```python
from build123d import *

# Parameters (mm, degrees)
SKETCH1_R           = 127.5
SKETCH1_R_2         = 110
BOSS_EXTRUDE1_DEPTH = 5
SKETCH4_R           = 1
CUT_EXTRUDE2_DEPTH  = 5
CIRPATTERN2_COUNT   = 4


with BuildPart() as part:
    # Sketch1 → Boss-Extrude1 (new body)
    with BuildSketch(Plane.XY):
        Circle(SKETCH1_R)
        Circle(SKETCH1_R_2, mode=Mode.SUBTRACT)
    extrude(amount=BOSS_EXTRUDE1_DEPTH)

    # Sketch4 → Cut-Extrude2 (cut)
    with BuildSketch(Plane.XY.offset(5)):
        with Locations((0, 125)):
            Circle(SKETCH4_R)
    cut_extrude2 = extrude(amount=-CUT_EXTRUDE2_DEPTH, mode=Mode.SUBTRACT)

    # CirPattern2: Cut-Extrude2 ×4 about axis
    cirpattern2_axis = Axis((0, 0, 0), (0, 0, 1))
    for i in range(1, CIRPATTERN2_COUNT):
        add(cut_extrude2.rotate(cirpattern2_axis, i * 360 / CIRPATTERN2_COUNT), mode=Mode.SUBTRACT)


solid = part.part
```
The listing builds one solid part. Answer for the finished solid, in the listing's coordinates (mm). Coordinates: 2 decimals unless noted, no trailing zeros. Write each loop counter-clockwise with the first axis right and the second up, starting at its lowest first coordinate (ties: lowest second). Pieces come first, ordered by that corner, then holes. Notation, with made-up numbers: (-13, 62.5) - (18, 62.5) arc R21 cw to (18, 81.5) - close; hole circle Ø8 at (-24.75, 2). An arc over 180 degrees is marked (long way). Return JSON: item names as keys, results as strings. Group by question number.
1. A cutting plane is placed at C-C, the plane y = 77. Determine the outline of the cut face in (x, z), plus the area to 3 significant figures.
2. Given pin 1 (1 mm diameter, centred on x = 14.5, z = 4, fed in from +Y); pin 2 (3 mm diameter, centred on y = 0.5, z = 4.5, fed in from -X); pin 3 (3 mm diameter, centred on y = 76, z = 1, fed in from +X), each flat-ended and moving along its own axis, determine where each tip first touches the part or whether it passes through.
3. A cutting plane is placed at A-A, the plane x = 38.5. Determine the outline of the cut face in (y, z), plus the area to 3 significant figures.
4. A cutting plane is placed at B-B, the plane z = 1.95. Determine the outline of the cut face in (x, y).
5. Straight lines are drawn through the part: L1, parallel to Y at x = 0, z = 2.1; L2, parallel to Y at x = -3.5, z = 1.4; L3, parallel to X at y = -75.5, z = 3.3. For each, find the intervals that lie inside material, in ascending order.
Ans:
{
 "1": {"outline": "(-101.62, 0) - (-78.56, 0) - (-78.56, 5) - (-101.62, 5) - close; (78.56, 0) - (101.62, 0) - (101.62, 5) - (78.56, 5) - close", "area": "231 mm²"},
 "2": {"pin 1": "y = 126.73", "pin 2": "x = -127.5", "pin 3": "x = 103.47"},
 "3": {"outline": "(-121.55, 0) - (-103.04, 0) - (-103.04, 5) - (-121.55, 5) - close; (103.04, 0) - (121.55, 0) - (121.55, 5) - (103.04, 5) - close", "area": "185 mm²"},
 "4": {"outline": "circle Ø255 at (0, 0); hole circle Ø2 at (-125, 0); hole circle Ø220 at (0, 0); hole circle Ø2 at (0, -125); hole circle Ø2 at (0, 125); hole circle Ø2 at (125, 0)"},
 "5": {"L1": "-127.5 to -126, -124 to -110, 110 to 124, 126 to 127.5", "L2": "-127.45 to -109.94, 109.94 to 127.45", "L3": "-102.74 to -80, 80 to 102.74"}
}
